```python
from build123d import *

# Parameters (mm, degrees)
SKETCH1_W                = 41
SKETCH1_H                = 4
SKETCH2_R                = 31
BOSS_EXTRUDE1_DEPTH      = 4
M52_CLEARANCE_HOLE1_D    = 57
F_7_0_7_DIAMETER_HOLE1_D = 7


with BuildPart() as part:
    # Sketch1 → Revolve1 (revolve)
    with BuildSketch(Plane.XY.offset(89.5), mode=Mode.PRIVATE) as revolve1_sk:
        with Locations((-1049.091991574, 72.472431577)):
            Rectangle(SKETCH1_W, SKETCH1_H)
    revolve(revolve1_sk.sketch.rotate(Axis((-1069.591991574, 74.472431577, 89.5), (0, -1, 0)), 270), axis=Axis((-1069.591991574, 74.472431577, 89.5), (0, -1, 0)))

    # Sketch2 → Boss-Extrude1 (add)
    with BuildSketch(Plane.XZ.offset(-70.472431577)):
        with Locations(Location((-1069.591991574, 89.5, 0), (0, 0, 270))):
            Circle(SKETCH2_R)
    extrude(amount=BOSS_EXTRUDE1_DEPTH)

    # M52 Clearance Hole1 (through all)
    with Locations(Plane(origin=(0, 66.472431577, 0), x_dir=(-1, 0, 0), z_dir=(0, -1, 0))):
        with Locations((1069.591991574, -89.5)):
            Hole(M52_CLEARANCE_HOLE1_D / 2)

    # Ø7.0 (7) Diameter Hole1 (through all)
    with Locations(Plane(origin=(0, 70.472431577, 0), x_dir=(-1, 0, 0), z_dir=(0, -1, 0))):
        with Locations((1069.591991574, -125.5), (1100.76890611, -107.5), (1100.76890611, -71.5), (1069.591991574, -53.5), (1038.415077038, -71.5), (1038.415077038, -107.5)):
            Hole(F_7_0_7_DIAMETER_HOLE1_D / 2)


solid = part.part
```
Work out the finished part from the listing and answer in its coordinate system (mm). A direction names the side the tool comes from. Give positions to 0.01 mm unless a question says otherwise; leave off trailing zeros. Loops run counter-clockwise (first coordinate to the right, second up) from the corner with the lowest first, then second, coordinate; pieces in that order, holes last. Notation, with made-up numbers: (61, 42) -> (111, 42) arc R29 ccw to (111, 69) -> close; hole circle Ø3 at (35, 34.25). An arc over 180 degrees is marked (long way). Use CSV: the item, a comma, the result in double quotes.
1. The mould has two halves that part along Z. Classify faces 1 (the flat face through (-1097, 70.472, 74)), 2 (the cylindrical face through (-1066.254, 72.5, 124.449)), 3 (the cylindrical face through (-1028.94, 72.5, 94.84)): +Z half, -Z half, draft (parallel to the pull), parting line (faces both ways), or undercut.
Found:
face 1,"draft"
face 2,"undercut"
face 3,"parting line"
2. The part is cut by section C-C (z = 72.5). Write down the section's boundary in (x, y), then the cut area to 3 significant figures.
Found:
outline,"(-1106.9, 70.47) -> (-1104.12, 70.47) -> (-1104.12, 74.47) -> (-1106.9, 74.47) -> close; (-1097.41, 70.47) -> (-1095.51, 70.47) -> (-1095.51, 66.47) -> (-1092.47, 66.47) -> (-1092.47, 74.47) -> (-1097.41, 74.47) -> close; (-1046.72, 66.47) -> (-1043.67, 66.47) -> (-1043.67, 70.47) -> (-1041.77, 70.47) -> (-1041.77, 74.47) -> (-1046.72, 74.47) -> close; (-1035.06, 70.47) -> (-1032.28, 70.47) -> (-1032.28, 74.47) -> (-1035.06, 74.47) -> close"
area,"86.2 mm^2"
3. The part is cut by section B-B (x = -1049). Write down the section's boundary in (y, z).
Found:
outline,"(66.47, 66.33) -> (70.47, 66.33) -> (70.47, 54.05) -> (74.47, 54.05) -> (74.47, 69.8) -> (66.47, 69.8) -> close; (66.47, 109.2) -> (74.47, 109.2) -> (74.47, 124.95) -> (70.47, 124.95) -> (70.47, 112.67) -> (66.47, 112.67) -> close"
4. The part is cut by section A-A (z = 89.5). Write down the section's boundary in (x, y).
Found:
outline,"(-1110.59, 70.47) -> (-1100.59, 70.47) -> (-1100.59, 66.47) -> (-1098.09, 66.47) -> (-1098.09, 74.47) -> (-1110.59, 74.47) -> close; (-1041.09, 66.47) -> (-1038.59, 66.47) -> (-1038.59, 70.47) -> (-1028.59, 70.47) -> (-1028.59, 74.47) -> (-1041.09, 74.47) -> close"
5. Flat-ended cylindrical pins translate along their axes: pin 1 Ø24.5 at (x, z) = (-1085.5, 101) entering from -Y; pin 2 Ø2 at (x, y) = (-1096.5, 72.5) entering from -Z; pin 3 Ø1.5 at (y, z) = (69.5, 63) entering from +X; pin 4 Ø1 at (x, y) = (-1094, 68) entering from +Z. Find the tip coordinate at first contact, or state that the pin passes through.
Found:
pin 1,"y = 66.47"
pin 2,"z = 57.72"
pin 3,"x = -1052.33"
pin 4,"z = 109.23"
6. A tool of negligible diameter and unlimited length cuts with its end or side. For faces 4 (the cylindrical face through (-1043.453, 68.5, 72.835)), 5 (the flat face through (-1095, 66.472, 76)), from which of +Z, -Z, +X, -X, +Y, -Y can it reach the whole face along a straight path? Write none if from no direction.
Found:
face 4,"-Y"
face 5,"+Z, -Z, +X, -X, -Y"
7. Straight lines are drawn through the part: line 1 (X direction, y = 73.05, z = 71.5); line 2 (Z direction, x = -1068.5, y = 71.5); line 3 (Z direction, x = -1040.5, y = 72.5). For each, find the intervals that lie inside material, in ascending order.
Found:
line 1,"-1106.43 to -1104.27, -1097.27 to -1091.69, -1047.5 to -1041.92, -1034.92 to -1032.75"
line 2,"48.51 to 50.17, 56.83 to 61.02, 117.98 to 122.17, 128.83 to 130.49"
line 3,"60.61 to 68.69, 74.31 to 104.69, 110.31 to 118.39"
8. The part is cut by section D-D (y = 72.25). Write down the section's boundary in (x, z).
Found:
outline,"circle Ø82 at (-1069.59, 89.5); hole circle Ø7 at (-1100.77, 71.5); hole circle Ø7 at (-1100.77, 107.5); hole circle Ø57 at (-1069.59, 89.5); hole circle Ø7 at (-1069.59, 53.5); hole circle Ø7 at (-1069.59, 125.5); hole circle Ø7 at (-1038.42, 71.5); hole circle Ø7 at (-1038.42, 107.5)"
